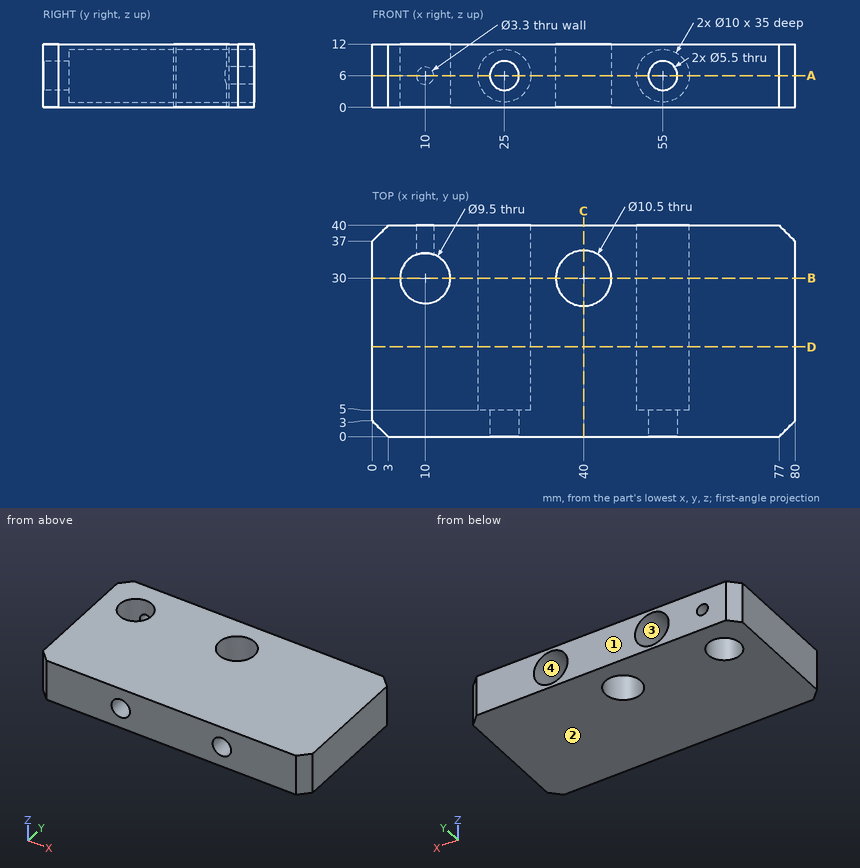
Here's the drawing with two shaded views (mm, measured from the low corner). I have some questions. Give positions to 0.01 mm unless a question says otherwise; leave off trailing zeros. Loops run counter-clockwise (first coordinate to the right, second up) from the corner with the lowest first, then second, coordinate; pieces in that order, holes last. Notation, with made-up numbers: (38, 0.25) -> (72, 0.25) arc R29 ccw to (72, 39.25) -> close; hole circle Ø6 at (-33, 23.25). An arc over 180 degrees is marked (long way). Answer as a JSON object with one key per item and string values. Group by question number.
Item 1: I need wall thicknesses on L1, parallel to Y at x = 10, z = 3.5; L2, parallel to Z at x = 10, y = 38.25; L3, parallel to X at y = 18, z = 4.25. Which ranges of each line are inside material? Lowest first, please.
Item 2: Imagine slicing it at A-A on z = 6. Give the number of separate pieces and of enclosed holes in the cut face, then the cut area to 3 significant figures.
Item 3: Imagine slicing it at D-D on y = 17. Write out the boundary of the cut face in (x, z).
Item 4: Imagine slicing it at C-C on x = 40. Write out the boundary of the cut face in (y, z).
Item 5: Thinking about a two-plate mould opening in Z: for the marked faces 1, 2, 3 and 4, which applies, pulls with the +Z half, pulls with the -Z half, needs draft (parallel to the pull), parting line crosses it, or undercut?
Item 6: Imagine slicing it at B-B on y = 30. Write out the boundary of the cut face in (x, z).
Item 7: Will these pins go through, and if not, where does the flat tip stop? pin 1 (12 mm diameter, centred on x = 40.5, y = 29.5, fed in from +Z); pin 2 (3.5 mm diameter, centred on x = 55, z = 6, fed in from -Y); pin 3 (5 mm diameter, centred on x = 26, z = 7.5, fed in from +Y); pin 4 (2.5 mm diameter, centred on x = 10, z = 6, fed in from +Y).
Answer list:
{
 "1": {"L1": "y = 0 to 25.25, 34.75 to 40", "L2": "z = 0 to 4.35, 7.65 to 12", "L3": "x = 0 to 20.32, 29.68 to 50.32, 59.68 to 80"},
 "2": {"separate pieces": "3", "enclosed holes": "1", "area": "2,250 mm2"},
 "3": {"outline": "(0, 0) -> (80, 0) -> (80, 12) -> (0, 12) -> close; hole circle Ø10 at (25, 6); hole circle Ø10 at (55, 6)"},
 "4": {"outline": "(0, 0) -> (24.75, 0) -> (24.75, 12) -> (0, 12) -> close; (35.25, 0) -> (40, 0) -> (40, 12) -> (35.25, 12) -> close"},
 "5": {"face 1": "needs draft", "face 2": "pulls with the -Z half", "face 3": "undercut", "face 4": "undercut"},
 "6": {"outline": "(0, 0) -> (5.25, 0) -> (5.25, 12) -> (0, 12) -> close; (14.75, 0) -> (34.75, 0) -> (34.75, 12) -> (14.75, 12) -> close; (45.25, 0) -> (80, 0) -> (80, 12) -> (45.25, 12) -> close; hole circle Ø10 at (25, 6); hole circle Ø10 at (55, 6)"},
 "7": {"pin 1": "stops at z = 12", "pin 2": "passes through", "pin 3": "stops at y = 5", "pin 4": "stops at y = 25.42"}
}
